Input: part model. Units: mm. Frame: model coordinates. A direction names the side the tool comes from. Give positions to 0.01 mm unless a question says otherwise; leave off trailing zeros. Loops run counter-clockwise (first coordinate to the right, second up) from the corner with the lowest first, then second, coordinate; pieces in that order, holes last. Notation, with made-up numbers: M -15,4.5 L 5,4.5 A37 cw 5,43.5 Z; hole C -28,-13 d4. An arc over 180 degrees is marked long. Use CSV: the item, a comma, the result in double quotes. Start each with the question number.
from build123d import *

# Parameters (mm, degrees)
SKETCH_1_W      = 724.5
SKETCH_1_H      = 1319
EXTRUDE_1_DEPTH = 28
SHELL_1_T       = -2
SKETCH_2_W      = 724.5
SKETCH_2_H      = 1319
SKETCH_2_W_2    = 684.5
SKETCH_2_H_2    = 1279
EXTRUDE_2_DEPTH = 2


with BuildPart() as part:
    # 草图1 → 凸台-拉伸1 (new body)
    with BuildSketch(Plane.XY):
        with Locations((362.25, 659.5)):
            Rectangle(SKETCH_1_W, SKETCH_1_H)
    extrude(amount=EXTRUDE_1_DEPTH)

    # 抽壳1
    shell_1_openings = [part.faces().sort_by_distance(p)[0] for p in [
        (362.25, 659.5, 28),
    ]]
    offset(amount=SHELL_1_T, openings=shell_1_openings, kind=Kind.INTERSECTION)

    # 草图2 → 凸台-拉伸2 (add)
    with BuildSketch(Plane.XY.offset(28)):
        with Locations((362.25, 659.5)):
            Rectangle(SKETCH_2_W, SKETCH_2_H)
        with Locations((362.25, 659.5)):
            Rectangle(SKETCH_2_W_2, SKETCH_2_H_2, mode=Mode.SUBTRACT)
    extrude(amount=-EXTRUDE_2_DEPTH)


solid = part.part
Item 1: Set-up query: faces 4 (the flat face through (0, 650, 14)), 5 (the flat face through (722.5, 650, 14)). Return all of +Z, -Z, +X, -X, +Y, -Y with unobstructed straight access to the full face (end or side cutting, diameter ignored); none if empty.
Item 2: First-contact query: pin 1 Ø6 at (x, y) = (467, 1036.5) entering from +Z. Flat tip, straight axial feed; report the tip coordinate or a pass-through.
Item 3: Section A-A (z = 17). Output: boundary loops of the cut face in (x, y), then the cut area to 3 significant figures.
Item 4: Mould query, pull axis Y, two halves, no side actions, for faces 1 (the flat face through (724.5, 650, 14)), 2 (the flat face through (2, 650, 14)), 3 (the flat face through (357, 1319, 14)). Classes: +Y half, -Y half, draft (parallel to the pull), parting line (faces both ways), or undercut.
Item 5: Material intervals for line 1 (Y direction, x = 605, z = 2.5); line 2 (X direction, y = 177, z = 22.75); line 3 (Y direction, x = 595.5, z = 26.5), sorted ascending.
Item 6: Section B-B (y = 1216.5). Output: boundary loops of the cut face in (x, z), then the cut area to 4 significant figures.
Item 7: Section C-C (x = 674). Output: boundary loops of the cut face in (y, z).
Recorded:
1,face 4,"+Z, -Z, -X, +Y, -Y"
1,face 5,"none"
2,pin 1,"z = 2"
3,outline,"M 0,0 L 724.5,0 L 724.5,1319 L 0,1319 Z; hole M 2,2 L 722.5,2 L 722.5,1317 L 2,1317 Z"
3,area,"8,160 mm²"
4,face 1,"draft"
4,face 2,"undercut"
4,face 3,"+Y half"
5,line 1,"0 to 2, 1317 to 1319"
5,line 2,"0 to 2, 722.5 to 724.5"
5,line 3,"0 to 20, 1299 to 1319"
6,outline,"M 0,0 L 724.5,0 L 724.5,28 L 704.5,28 L 704.5,26 L 722.5,26 L 722.5,2 L 2,2 L 2,26 L 20,26 L 20,28 L 0,28 Z"
6,area,"1,625 mm²"
7,outline,"M 0,0 L 1319,0 L 1319,28 L 1299,28 L 1299,26 L 1317,26 L 1317,2 L 2,2 L 2,26 L 20,26 L 20,28 L 0,28 Z"
